Geometry check sheet. Reference: the model listing, model coordinates, mm. A direction names the side the tool comes from. Give positions to 0.01 mm unless a question says otherwise; leave off trailing zeros. Loops run counter-clockwise (first coordinate to the right, second up) from the corner with the lowest first, then second, coordinate; pieces in that order, holes last. Notation, with made-up numbers: (17, 38.25) -> (57, 38.25) arc R21 cw to (57, 74.25) -> close; hole circle Ø6 at (-35, 65.25). An arc over 180 degrees is marked (long way). Answer as a JSON object with one key per item and string values.
from build123d import *

# Parameters (mm, degrees)
SKETCH1_R           = 27.5
BOSS_EXTRUDE1_DEPTH = 11
SKETCH2_R           = 13.5
BOSS_EXTRUDE2_DEPTH = 3.5
SKETCH3_R           = 15
BOSS_EXTRUDE3_DEPTH = 14.5
SKETCH4_R           = 14
BOSS_EXTRUDE4_DEPTH = 19
SKETCH5_R           = 15
BOSS_EXTRUDE5_DEPTH = 49
SKETCH6_R           = 9
CUT_EXTRUDE1_DEPTH  = 52
SKETCH7_R           = 10
CUT_EXTRUDE2_DEPTH  = 38
SKETCH8_R           = 5.5
CUT_EXTRUDE3_DEPTH  = 6.5
SKETCH9_R           = 3.25
CUT_EXTRUDE4_DEPTH  = 6.5
CIRPATTERN1_COUNT   = 3
SKETCH10_R          = 4
CUT_EXTRUDE5_DEPTH  = 26.75


with BuildPart() as part:
    # Sketch1 → Boss-Extrude1 (new body)
    with BuildSketch(Plane.XY):
        Circle(SKETCH1_R)
    extrude(amount=BOSS_EXTRUDE1_DEPTH)

    # Sketch2 → Boss-Extrude2 (add)
    with BuildSketch(Plane.XY.offset(11)):
        Circle(SKETCH2_R)
    extrude(amount=BOSS_EXTRUDE2_DEPTH)

    # Sketch3 → Boss-Extrude3 (add)
    with BuildSketch(Plane.XY.offset(14.5)):
        with Locations(Location((0, 0, 0), (0, 0, 180))):
            Circle(SKETCH3_R)
    extrude(amount=BOSS_EXTRUDE3_DEPTH)

    # Sketch4 → Boss-Extrude4 (add)
    with BuildSketch(Plane.XY.offset(29)):
        Circle(SKETCH4_R)
    extrude(amount=BOSS_EXTRUDE4_DEPTH)

    # Sketch5 → Boss-Extrude5 (add)
    with BuildSketch(Plane.XY.offset(48)):
        with Locations(Location((0, 0, 0), (0, 0, 180))):
            Circle(SKETCH5_R)
    extrude(amount=BOSS_EXTRUDE5_DEPTH)

    # Sketch6 → Cut-Extrude1 (cut)
    with BuildSketch(Plane.XY.offset(97)):
        Circle(SKETCH6_R)
    extrude(amount=-CUT_EXTRUDE1_DEPTH, mode=Mode.SUBTRACT)

    # Sketch7 → Cut-Extrude2 (cut)
    with BuildSketch(Plane.XY.offset(45)):
        Circle(SKETCH7_R)
    extrude(amount=-CUT_EXTRUDE2_DEPTH, mode=Mode.SUBTRACT)

    # Sketch8 → Cut-Extrude3 (cut)
    with BuildSketch(Plane(origin=(0, 0, 0), x_dir=(-1, 0, 0), z_dir=(0, 0, -1))):
        with Locations((0, 20)):
            Circle(SKETCH8_R)
    cut_extrude3 = extrude(amount=-CUT_EXTRUDE3_DEPTH, mode=Mode.SUBTRACT)

    # Sketch9 → Cut-Extrude4 (cut)
    with BuildSketch(Plane(origin=(0, 0, 6.5), x_dir=(-1, 0, 0), z_dir=(0, 0, -1))):
        with Locations((0, 20)):
            Circle(SKETCH9_R)
    cut_extrude4 = extrude(amount=-CUT_EXTRUDE4_DEPTH, mode=Mode.SUBTRACT)

    # CirPattern1: Cut-Extrude3, Cut-Extrude4 ×3 about axis
    cirpattern1_axis = Axis((0, 0, 0), (0, 0, 1))
    add([cut_extrude3.rotate(cirpattern1_axis, i * 360 / CIRPATTERN1_COUNT) for i in range(1, CIRPATTERN1_COUNT)], mode=Mode.SUBTRACT)
    add([cut_extrude4.rotate(cirpattern1_axis, i * 360 / CIRPATTERN1_COUNT) for i in range(1, CIRPATTERN1_COUNT)], mode=Mode.SUBTRACT)

    # Sketch10 → Cut-Extrude5 (cut, symmetric)
    with BuildSketch(Plane(origin=(0, 0, 0), x_dir=(1, 0, 0), z_dir=(0, 1, 0))):
        with Locations(Location((0, -34, 0), (0, 0, 270))):
            Circle(SKETCH10_R)
    extrude(amount=CUT_EXTRUDE5_DEPTH, both=True, mode=Mode.SUBTRACT)


solid = part.part
1) Section check D-D on y = 20. Record the cut outline in (x, z), plus the area to 3 significant figures.
Geometry check:
{"outline": "(-18.87, 0) -> (-5.5, 0) -> (-5.5, 6.5) -> (-3.25, 6.5) -> (-3.25, 11) -> (-18.87, 11) -> close; (3.25, 6.5) -> (5.5, 6.5) -> (5.5, 0) -> (18.87, 0) -> (18.87, 11) -> (3.25, 11) -> close", "area": "314 mm2"}
2) Tool access check on faces 4 (the face through (-2.93, -13.18, 12.73)), 5 (the face through (-8.06, -12.65, 21.65)), 6 (the face through (12.24, -12.11, 3.2)), 7 (the face through (-3.549, -11.549, 35.846)). Record the directions out of +Z, -Z, +X, -X, +Y, -Y that give a thin tool (end or side, any length) a straight path to the whole face; none if there is none.
Geometry check:
{"face 4": "none", "face 5": "+Z", "face 6": "-Z", "face 7": "+Y, -Y"}
3) Section check C-C on z = 12. Record the cut outline in (x, y), plus the area to 3 significant figures.
Geometry check:
{"outline": "circle Ø27 at (0, 0); hole circle Ø20 at (0, 0)", "area": "258 mm2"}
4) Section check B-B on y = 0. Record the cut outline in (x, z).
Geometry check:
{"outline": "(-27.5, 0) -> (27.5, 0) -> (27.5, 11) -> (13.5, 11) -> (13.5, 14.5) -> (15, 14.5) -> (15, 29) -> (14, 29) -> (14, 48) -> (15, 48) -> (15, 97) -> (9, 97) -> (9, 45) -> (10, 45) -> (10, 7) -> (-10, 7) -> (-10, 45) -> (-9, 45) -> (-9, 97) -> (-15, 97) -> (-15, 48) -> (-14, 48) -> (-14, 29) -> (-15, 29) -> (-15, 14.5) -> (-13.5, 14.5) -> (-13.5, 11) -> (-27.5, 11) -> close"}
5) Material ranges on line 1 along Z through (x, y) = (-6, -12.5); line 2 along Z through (x, y) = (0, -11.75); line 3 along Y through (x, z) = (0, 75.5), recorded low to high. Write a range as from..to.
Geometry check:
{"line 1": "z = 0..11, 14.5..97", "line 2": "z = 0..30, 38..97", "line 3": "y = -15..-9, 9..15"}
6) Depth check by flat-ended pin: P1, Ø1.5, axis at y = -0.5, z = 57, coming from the -X side; P2, Ø22, axis at x = 5, y = -2, coming from the +Z side; P3, Ø13, axis at x = 0, z = 34, coming from the +Y side; P4, Ø1.5, axis at y = 10, z = 19.5, coming from the -X side. Enter the tip coordinate at first touch or a pass-through.
Geometry check:
{"P1": "stops at x = -15", "P2": "stops at z = 97", "P3": "stops at y = 15", "P4": "stops at x = -11.81"}
7) Draft check along Y on faces 1 (the face through (0, 0, 0)), 2 (the face through (-8.06, -12.65, 72.16)), 3 (the face through (-9, 2, 45)). Enter one of: pulls with the +Y half, pulls with the -Y half, needs draft (parallel to the pull), parting line crosses it, or undercut.
Geometry check:
{"face 1": "needs draft", "face 2": "parting line crosses it", "face 3": "undercut"}
8) Section check A-A on x = -19. Record the cut outline in (y, z).
Geometry check:
{"outline": "(-19.88, 0) -> (-15.24, 0) -> (-15.24, 6.5) -> (-12.78, 6.5) -> (-12.78, 11) -> (-19.88, 11) -> close; (-7.22, 6.5) -> (-4.76, 6.5) -> (-4.76, 0) -> (19.88, 0) -> (19.88, 11) -> (-7.22, 11) -> close"}
